Check sheet for the modelled part. Datum: model origin and axes. Units: mm. A direction names the side the tool comes from. Coordinates: 2 decimals unless noted, no trailing zeros. Loops run counter-clockwise (first coordinate to the right, second up) from the corner with the lowest first, then second, coordinate; pieces in that order, holes last. Notation, with made-up numbers: (-5, 66.5) -> (49, 66.5) arc R28 cw to (49, 104.5) -> close; hole circle Ø6 at (30.5, -22). An arc over 180 degrees is marked (long way). Use one line per item in the form item = value.
from build123d import *


with BuildPart() as part:
    # Sketch1 → Revolve1 (revolve)
    with BuildSketch(Plane.XY, mode=Mode.PRIVATE) as revolve1_sk:
        Polygon((-17.760797342, 0), (-17.760797342, -2), (-11.760797342, -2), (-11.760797342, -3.125), (15.239202658, -3.125), (15.239202658, -5), (19.239202658, -5), (19.239202658, 0), align=None)
    revolve(revolve1_sk.sketch.rotate(Axis((-26.641196013, 0, 0), (1, 0, 0)), 270), axis=Axis((-26.641196013, 0, 0), (1, 0, 0)))


solid = part.part
(1) Scan lines: line 1 along X through (y, z) = (-2.25, 2.25); line 2 along X through (y, z) = (3, -0.75); line 3 along Z through (x, y) = (-10, 1.5). Record each from-to range of solid material in increasing order.
Established:
line_1 = 15.24 to 19.24
line_2 = -11.76 to 19.24
line_3 = -2.74 to 2.74
(2) Section check D-D, the plane z = -3.5. Record the boundary of the cut face in (x, y).
Established:
outline = (15.24, -3.57) -> (19.24, -3.57) -> (19.24, 3.57) -> (15.24, 3.57) -> close
(3) Section check C-C, the plane x = 1. Record the boundary of the cut face in (y, z) (3 decimals).
Established:
outline = circle Ø6.25 at (0, 0)
(4) Tool access check on faces 1 (the flat face through (19.239, 0, 0)), 2 (the cylindrical face through (1.93, -0.94, 2.98)). Record the directions out of +Z, -Z, +X, -X, +Y, -Y that give a thin tool (end or side, any length) a straight path to the whole face; none if there is none.
Established:
face_1 = +Z, -Z, +X, +Y, -Y
face_2 = -X
(5) Go/stop test with flat-tipped pins: P1, Ø4, axis at x = -13.5, z = 3, coming from the -Y side; P2, Ø2, axis at x = 13, z = 0.5, coming from the -Y side (3 decimals); P3, Ø1, axis at x = -4, z = 3, coming from the -Y side (3 decimals). Record where each tip stops, or that it passes through.
Established:
P1 = -2.39
P2 = -3.125
P3 = -1.875
(6) Section check A-A, the plane z = 0. Record the boundary of the cut face in (x, y) (3 decimals).
Established:
outline = (-17.761, -2) -> (-11.761, -2) -> (-11.761, -3.125) -> (15.239, -3.125) -> (15.239, -5) -> (19.239, -5) -> (19.239, 5) -> (15.239, 5) -> (15.239, 3.125) -> (-11.761, 3.125) -> (-11.761, 2) -> (-17.761, 2) -> close
